```python
from build123d import *

# Parameters (mm, degrees)
CRANK_WEB_DEPTH       = 10
SKETCH1_4_R           = 12.5
MAIN_JOURNAL_DEPTH    = 30
CRANK_PIN_SKETCH_25_R = 12.5
CRANK_PIN_25_DEPTH    = 50


with BuildPart() as part:
    # Crank Web Profile → Crank Web (new body)
    with BuildSketch(Plane.XY):
        with BuildLine():
            Line((-28.136908189, 0), (-44.72135955, 0))
            ThreePointArc((-44.72135955, 0), (-48.448139512, -1.666666667), (-49.6903995, -5.555555556))
            ThreePointArc((-49.6903995, -5.555555556), (0, -50), (49.6903995, -5.555555556))
            ThreePointArc((49.6903995, -5.555555556), (48.448139512, -1.666666667), (44.72135955, 0))
            Line((44.72135955, 0), (28.136908189, 0))
            ThreePointArc((28.136908189, 0), (24.92297014, 1.169777784), (23.212869424, 4.131759112))
            Line((23.212869424, 4.131759112), (17.234135678, 38.038843109))
            ThreePointArc((17.234135678, 38.038843109), (0, 52.5), (-17.234135678, 38.038843109))
            Line((-17.234135678, 38.038843109), (-23.212869424, 4.131759112))
            ThreePointArc((-23.212869424, 4.131759112), (-24.92297014, 1.169777784), (-28.136908189, 0))
        make_face()
    crank_web = extrude(amount=-CRANK_WEB_DEPTH)

    # Sketch1_4 → Main Journal (add)
    with BuildSketch(Plane.XY):
        Circle(SKETCH1_4_R)
    main_journal = extrude(amount=-MAIN_JOURNAL_DEPTH)

    # Crank Pin Sketch _25 → Crank Pin _25 (add)
    with BuildSketch(Plane.XY):
        with Locations((0, 35)):
            Circle(CRANK_PIN_SKETCH_25_R)
    extrude(amount=CRANK_PIN_25_DEPTH)

    # Mirror Web and Journal: Crank Web, Main Journal across plane
    add(crank_web.mirror(Plane.XY.offset(25)))
    add(main_journal.mirror(Plane.XY.offset(25)))


solid = part.part
```
The listing builds one solid part. Answer for the finished solid, in the listing's coordinates (mm). A direction names the side the tool comes from. Give positions to 0.01 mm unless a question says otherwise; leave off trailing zeros. Order: outer loops, then holes, each group sorted by start corner. A loop starts at its lowest first (then second) coordinate and runs counter-clockwise, first axis right, second up. Notation, with made-up numbers: (18, -39) - (46, -39) arc R11 cw to (46, -27) - close; hole circle Ø8 at (-30, -20). An arc over 180 degrees is marked (long way). Answer in a Markdown table with one row per item. Add a question column.
Q1. The part is cut by section B-B (z = 54). Determine the outline of the cut face in (x, y).
Q2. Which of the six approach directions +Z, -Z, +X, -X, +Y, -Y give full straight-line access (tool end or side, diameter ignored) to faces 5 (the cylindrical face through (-1.02, -49.99, 54.93)), 6 (the flat face through (-36, 0, -5)), 7 (the cylindrical face through (11.923, 3.755, 69.86))?
Q3. Given P1, Ø8, axis at x = 29.5, y = 9, coming from the -Z side; P2, Ø11, axis at x = -33, z = -6, coming from the +Y side; P3, Ø12, axis at x = -18, y = -21, coming from the +Z side; P4, Ø5, axis at x = 25.5, y = -7, coming from the -Z side, each flat-ended and moving along its own axis, determine where each tip first touches the part or whether it passes through.
Q4. The part is cut by section D-D (x = 0). Determine the outline of the cut face in (y, z).
Q5. The part is cut by section A-A (x = 30). Determine the outline of the cut face in (y, z).
Q6. Find the intervals of material crossed by line 1 along Z through (x, y) = (35, -1.5); line 2 along Z through (x, y) = (-3, -3); line 3 along Z through (x, y) = (4, 26), in increasing order. Write a range as [from, to].
Q7. The part is cut by section C-C (y = -39). Determine the outline of the cut face in (x, z), then the cut area to 3 significant figures.
Q8. For a pull along Z with two mould halves and no side action, classify faces 1 (the flat face through (0, 0, -30)), 2 (the flat face through (-1, -9, 0)), 3 (the cylindrical face through (-2.71, 22.797, 24.65)), 4 (the cylindrical face through (-24.89, 1.2, -4.93)) as released by +Z, released by -Z, zero draft, split by the parting line, or undercut.
Determined:
| question | item | result |
|---|---|---|
| 1 | outline | (-49.69, -5.56) arc R50 ccw to (49.69, -5.56) arc R5 ccw to (44.72, 0) - (28.14, 0) arc R5 cw to (23.21, 4.13) - (17.23, 38.04) arc R17.5 ccw to (-17.23, 38.04) - (-23.21, 4.13) arc R5 cw to (-28.14, 0) - (-44.72, 0) arc R5 ccw to start |
| 2 | face 5 | +Z, -Z, -Y |
| 2 | face 6 | +Z, -Z, -X, +Y |
| 2 | face 7 | +Z |
| 3 | P1 | passes through |
| 3 | P2 | stops at y = 0.04 |
| 3 | P3 | stops at z = 60 |
| 3 | P4 | stops at z = -10 |
| 4 | outline | (-50, -10) - (-12.5, -10) - (-12.5, -30) - (12.5, -30) - (12.5, -10) - (52.5, -10) - (52.5, 0) - (47.5, 0) - (47.5, 50) - (52.5, 50) - (52.5, 60) - (12.5, 60) - (12.5, 80) - (-12.5, 80) - (-12.5, 60) - (-50, 60) - (-50, 50) - (22.5, 50) - (22.5, 0) - (-50, 0) - close |
| 5 | outline | (-40, -10) - (0, -10) - (0, 0) - (-40, 0) - close; (-40, 50) - (0, 50) - (0, 60) - (-40, 60) - close |
| 6 | line 1 | z = [-10, 0], [50, 60] |
| 6 | line 2 | z = [-30, 0], [50, 80] |
| 6 | line 3 | z = [-10, 60] |
| 7 | outline | (-31.29, -10) - (31.29, -10) - (31.29, 0) - (-31.29, 0) - close; (-31.29, 50) - (31.29, 50) - (31.29, 60) - (-31.29, 60) - close |
| 7 | area | 1,250 mm² |
| 8 | face 1 | released by -Z |
| 8 | face 2 | undercut |
| 8 | face 3 | undercut |
| 8 | face 4 | zero draft |
